Geometry: see drawing. Coordinates: mm, zero at the bounding-box minimum. A direction names the side the tool comes from. Round coordinates to 2 decimals unless told otherwise and drop trailing zeros. Order: outer loops, then holes, each group sorted by start corner. A loop starts at its lowest first (then second) coordinate and runs counter-clockwise, first axis right, second up. Notation, with made-up numbers: (38.5, 29.25) -> (90.5, 29.25) arc R17 ccw to (90.5, 34.25) -> close; hole circle Ø10 at (-31, -12.75). An arc over 180 degrees is marked (long way). One line per item, written item: value. Start each with the question number.
1) Section D-D (z = 21). Return the cut outline in (x, y).
2) Section C-C (y = 14). Return the cut outline in (x, z), and give its area (3 significant figures).
3) Section A-A (x = 15). Return the cut outline in (y, z).
4) Ray query, L1, parallel to Y at x = 27.5, z = 13.5; L2, parallel to Z at x = 15.25, y = 7; L3, parallel to X at y = 97, z = 23.25. Return the intervals inside material, ascending.
5) Pin query (flat end, axial travel): P1, Ø1, axis at x = 21, z = 7, coming from the +Y side; P2, Ø1, axis at x = 4, z = 21, coming from the -Y side; P3, Ø1.5, axis at x = 18.5, y = 49.5, coming from the +Z side. Return the tip coordinate at first contact, or that it passes through.
6) Reachability of the marked faces 4 and 5 from +Z, -Z, +X, -X, +Y, -Y: full face, straight path, thin tool, end or side. Return the list, or none.
7) Mould query, pull axis Y, two halves, no side actions, for the marked faces 1, 2 and 3. Classes: pulls with the +Y half, pulls with the -Y half, needs draft (parallel to the pull), parting line crosses it, or undercut.
8) Section B-B (z = 15). Return the cut outline in (x, y).
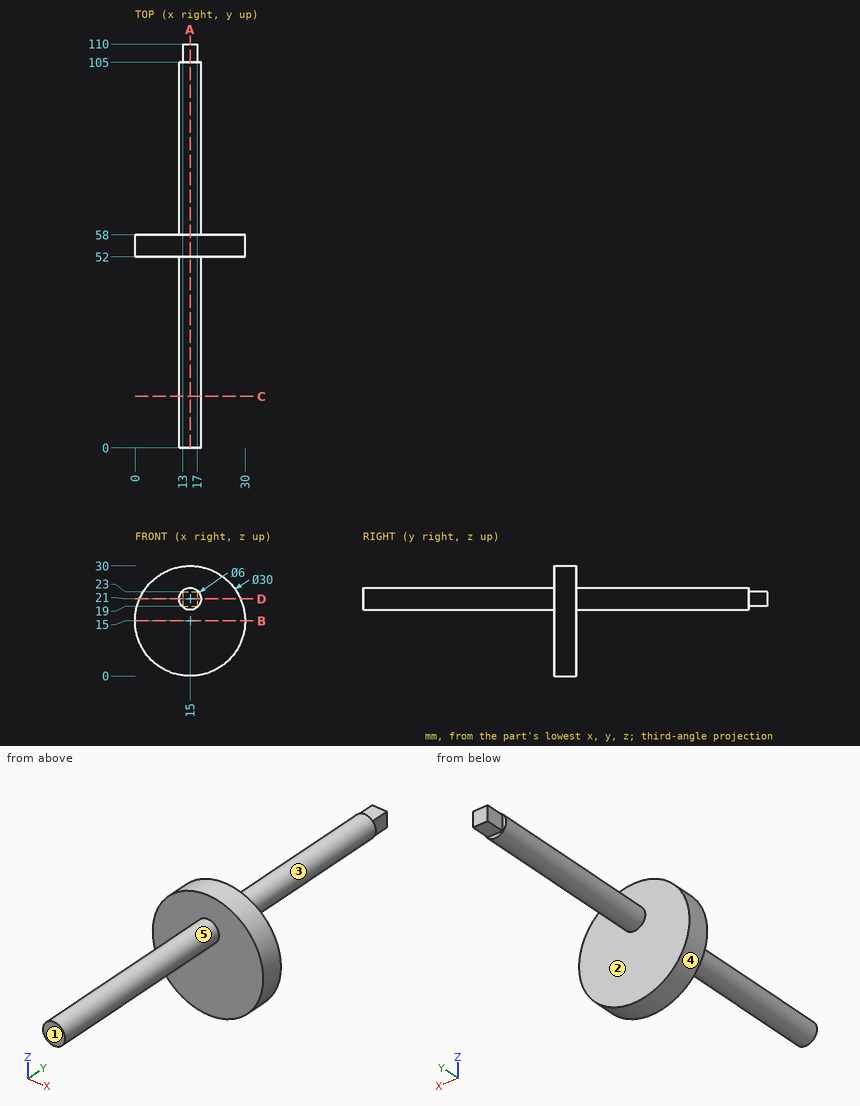
Findings:
1. outline: (1.25, 52) -> (12, 52) -> (12, 0) -> (18, 0) -> (18, 52) -> (28.75, 52) -> (28.75, 58) -> (18, 58) -> (18, 105) -> (17, 105) -> (17, 110) -> (13, 110) -> (13, 105) -> (12, 105) -> (12, 58) -> (1.25, 58) -> close
2. outline: circle Ø6 at (15, 21)
2. area: 28.3 mm2
3. outline: (0, 18) -> (52, 18) -> (52, 0) -> (58, 0) -> (58, 18) -> (105, 18) -> (105, 19) -> (110, 19) -> (110, 23) -> (105, 23) -> (105, 24) -> (58, 24) -> (58, 30) -> (52, 30) -> (52, 24) -> (0, 24) -> close
4. L1: 52 to 58
4. L2: 18.01 to 23.99
4. L3: 13.02 to 16.98
5. P1: y = 58
5. P2: y = 52
5. P3: z = 22.2
6. face 4: +Y, -Y
6. face 5: -Y
7. face 1: pulls with the -Y half
7. face 2: pulls with the +Y half
7. face 3: needs draft
8. outline: (0, 52) -> (30, 52) -> (30, 58) -> (0, 58) -> close
